Could you check a few things on this model? Use its own coordinates, in mm. Give positions to 0.01 mm unless a question says otherwise; leave off trailing zeros. Write each loop counter-clockwise with the first axis right and the second up, starting at its lowest first coordinate (ties: lowest second). Pieces come first, ordered by that corner, then holes. Notation, with made-up numbers: M -2,-26.75 L 54,-26.75 A12 ccw 54,-17.75 Z; hole C 69.25,-26 d2. An arc over 180 degrees is marked long. Write each question's results on one line, items separated by ' | '. Start each with the question number.
from build123d import *


with BuildPart() as part:
    # Sweep1: sweep along a path in Sketch1
    with BuildLine(Plane.XY) as sweep1_path:
        Line((-280, 48.55), (280, 48.55))
        ThreePointArc((280, 48.55), (328.55, 0), (280, -48.55))
        Line((280, -48.55), (-280, -48.55))
        ThreePointArc((-280, -48.55), (-328.55, 0), (-280, 48.55))
    # Sketch2 → Sweep1 (sweep)
    with BuildSketch(Plane(origin=(0, 0, 0), x_dir=(1, 0, 0), z_dir=(0, 1, 0))):
        Polygon((-328.55, 2.5), (-328.55, -2.5), (-340.05, -6.5), (-340.05, 6.5), align=None)
    sweep(path=sweep1_path.line)


solid = part.part
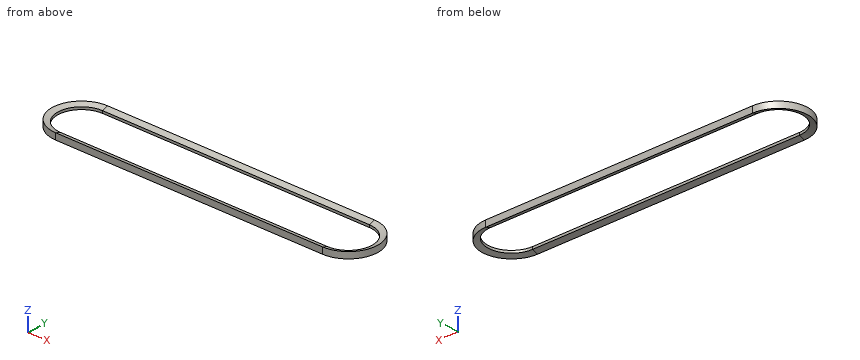
Q1. Please list where these lines run through material, in increasing order: line 1 (Y direction, x = 157.5, z = 0.5); line 2 (X direction, y = 35, z = -2); line 3 (X direction, y = -28, z = -1.5). Write a range as [from, to].
Q2. If we section it at A-A (y = 0): Please give me the cut outline in (x, z), plus the area to 3 significant figures.
Q3. If we section it at B-B (x = 93): Please give me the cut outline in (y, z).
Q4. I'm going to push a flat-ended pin straight in: P1, Ø6, axis at y = -16.5, z = 1.5, coming from the +X side. Where does the tip first touch, or does it pass through?
Determined:
1) line 1: y = [-60.05, -48.55], [48.55, 60.05] | line 2: x = [-328.8, -313.65], [313.65, 328.8] | line 3: x = [-333.12, -319.66], [319.66, 333.12]
2) outline: M -340.05,-6.5 L -328.55,-2.5 L -328.55,2.5 L -340.05,6.5 Z; M 328.55,-2.5 L 340.05,-6.5 L 340.05,6.5 L 328.55,2.5 Z | area: 207 mm²
3) outline: M -60.05,-6.5 L -48.55,-2.5 L -48.55,2.5 L -60.05,6.5 Z; M 48.55,-2.5 L 60.05,-6.5 L 60.05,6.5 L 48.55,2.5 Z
4) P1: stops at x = 338.51
